Input: part model. Units: mm. Frame: model coordinates. A direction names the side the tool comes from. Give positions to 0.01 mm unless a question says otherwise; leave off trailing zeros. Loops run counter-clockwise (first coordinate to the right, second up) from the corner with the lowest first, then second, coordinate; pieces in that order, holes last. Notation, with made-up numbers: M 50.5,51.5 L 65.5,51.5 A27 cw 65.5,88.5 Z; hole C 32.5,53 d8. An arc over 180 degrees is marked long. Answer as a JSON object with one key per item and string values. Group by question number.
```python
from build123d import *

# Parameters (mm, degrees)
PLATE_PROFILE_SKETCH_R    = 6.5
MOUNTING_PLATE_11MM_DEPTH = 11
SUPPORT_BLOCK_37MM_DEPTH  = 37
FILLET_R10_R              = 10
ARM_HOLE_DEPTH            = 124.555655476
ARM_HOLE_DEPTH_BACK       = 124.555655476
ARM_HOLE_SKETCH_R         = 12


with BuildPart() as part:
    # Plate Profile Sketch → Mounting Plate 11mm (new body)
    with BuildSketch(Plane(origin=(0, 0, 0), x_dir=(1, 0, 0), z_dir=(0, 1, 0))):
        with BuildLine():
            Line((-15, 0), (-15, 64))
            Line((-15, 64), (-32, 64))
            Line((-32, 64), (-32, 99))
            Line((-32, 99), (-21, 99))
            Line((-21, 99), (-21, 82))
            Line((-21, 82), (21, 82))
            Line((21, 82), (21, 98.934064449))
            Line((21, 98.934064449), (32, 98.934064449))
            Line((32, 98.934064449), (32, 64))
            Line((32, 64), (15, 64))
            Line((15, 64), (15, 0))
            ThreePointArc((15, 0), (0, -15), (-15, 0))
        make_face()
        with Locations(Location((0, 0, 0), (0, 0, 270))):
            Circle(PLATE_PROFILE_SKETCH_R, mode=Mode.SUBTRACT)
        with Locations(Location((0, 30, 0), (0, 0, 270))):
            Circle(PLATE_PROFILE_SKETCH_R, mode=Mode.SUBTRACT)
    extrude(amount=MOUNTING_PLATE_11MM_DEPTH)

    # Support Block Sketch → Support Block 37mm (add)
    with BuildSketch(Plane.XZ):
        Polygon((-32, -64), (32, -64), (32, -98.934064449), (21, -98.934064449), (21, -82), (-21, -82), (-21, -99), (-32, -99), align=None)
    extrude(amount=SUPPORT_BLOCK_37MM_DEPTH)

    # Fillet R10
    fillet_r10_edges = [part.edges().sort_by_distance(p)[0] for p in [
        (-15, 5.5, -64),
        (15, 5.5, -64),
    ]]
    fillet(fillet_r10_edges, radius=FILLET_R10_R)

    # Arm Hole Sketch → Arm Hole (cut, two sides: drawn at the far end of the back side and taken through both)
    with BuildSketch(Plane(origin=(32, 0, 0), x_dir=(0, 0, -1), z_dir=(1, 0, 0)).offset(-ARM_HOLE_DEPTH_BACK)):
        with Locations((98.934064449, -11)):
            Circle(ARM_HOLE_SKETCH_R)
    extrude(amount=ARM_HOLE_DEPTH + ARM_HOLE_DEPTH_BACK, mode=Mode.SUBTRACT)


solid = part.part
```
1. Section A-A (x = 0). Output: boundary loops of the cut face in (y, z), then the cut area to 3 significant figures.
2. Section B-B (z = -30). Output: boundary loops of the cut face in (x, y).
3. Mould query, pull axis X, two halves, no side actions, for faces 1 (the flat face through (0, -13, -82)), 2 (the flat face through (27, 6, -98.934)), 3 (the flat face through (15, 5, -27)), 4 (the flat face through (-32, -13, -82)). Classes: pulls with the +X half, pulls with the -X half, needs draft (parallel to the pull), parting line crosses it, or undercut.
4. Reachability of faces 5 (the flat face through (32, -13, -81)), 6 (the flat face through (-21, -12.7, -86.6)), 7 (the flat face through (-5, 0, -25)), 8 (the flat face through (-15, 5, -27)), 9 (the cylindrical face through (18.01, 5.58, -61.15)) from +Z, -Z, +X, -X, +Y, -Y: full face, straight path, thin tool, end or side. Return the list, or none.
5. First-contact query: P1, Ø12, axis at x = -17.5, y = -2, coming from the -Z side; P2, Ø5.5, axis at x = 27.5, y = -32.5, coming from the -Z side; P3, Ø12, axis at x = -8, y = -7.5, coming from the -Z side; P4, Ø5, axis at y = -9, z = -90, coming from the -X side. Flat tips, straight axial feed; report the tip coordinate or a pass-through.
6. Section C-C (y = -28.5). Output: boundary loops of the cut face in (x, z).
7. Material intervals for L1, parallel to X at y = -8, z = -86; L2, parallel to X at y = 7, z = -30; L3, parallel to Z at x = -10, y = -30, sorted ascending.
8. Section D-D (z = -88.5). Output: boundary loops of the cut face in (x, y).
Geometry results:
{
 "1": {"outline": "M -37,-82 L 11,-82 L 11,-36.5 L 0,-36.5 L 0,-64 L -37,-64 Z; M 0,-23.5 L 11,-23.5 L 11,-6.5 L 0,-6.5 Z; M 0,6.5 L 11,6.5 L 11,15 L 0,15 Z", "area": "1,450 mm2"},
 "2": {"outline": "M -15,0 L -6.5,0 L -6.5,11 L -15,11 Z; M 6.5,0 L 15,0 L 15,11 L 6.5,11 Z"},
 "3": {"face 1": "undercut", "face 2": "needs draft", "face 3": "pulls with the +X half", "face 4": "pulls with the -X half"},
 "4": {"face 5": "+Z, -Z, +X, +Y, -Y", "face 6": "-Z, +Y, -Y", "face 7": "+Z, +X, -X, -Y", "face 8": "+Z, -X, +Y, -Y", "face 9": "+Z, +X, +Y, -Y"},
 "5": {"P1": "z = -99", "P2": "z = -98.93", "P3": "z = -82", "P4": "through"},
 "6": {"outline": "M -32,-99 L -21,-99 L -21,-82 L 21,-82 L 21,-98.93 L 32,-98.93 L 32,-64 L -32,-64 Z"},
 "7": {"L1": "-32 to -21, 21 to 32", "L2": "-15 to -6.5, 6.5 to 15", "L3": "-82 to -64"},
 "8": {"outline": "M -32,-37 L -21,-37 L -21,-16.93 L -32,-16.93 Z; M -32,-5.07 L -21,-5.07 L -21,11 L -32,11 Z; M 21,-37 L 32,-37 L 32,-16.93 L 21,-16.93 Z; M 21,-5.07 L 32,-5.07 L 32,11 L 21,11 Z"}
}
